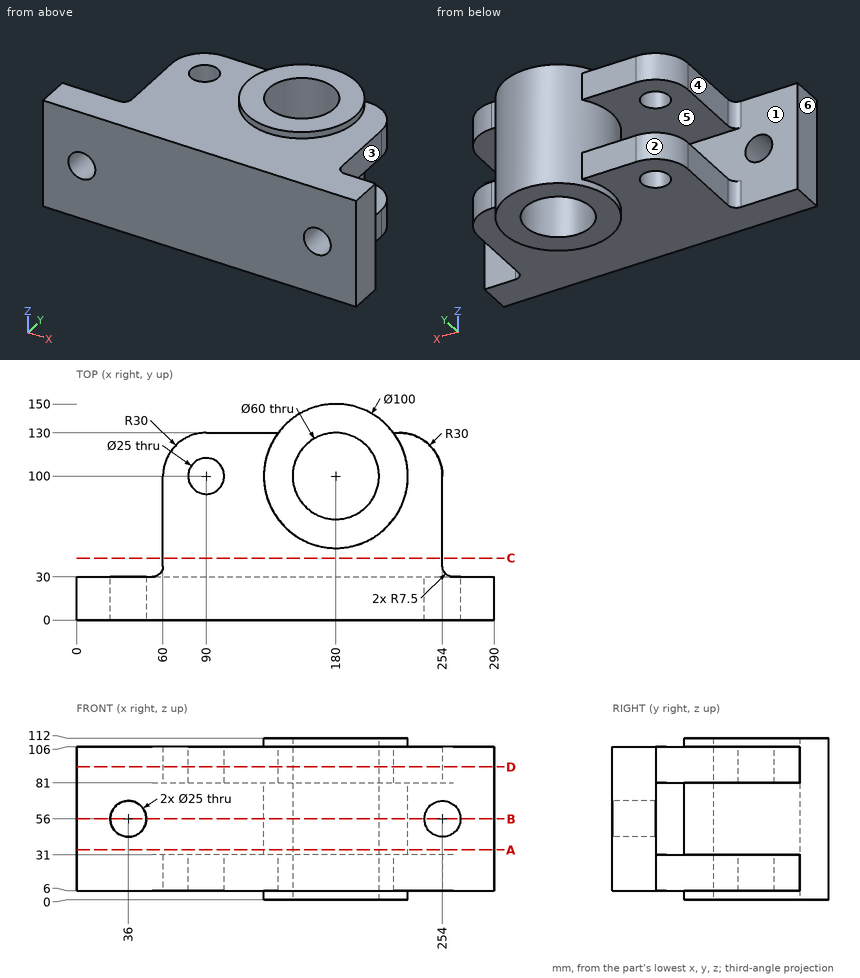
For this review, use the dimensioned drawing (mm, ordinates from the lowest corner) and the shaded views. A direction names the side the tool comes from. Give positions to 0.01 mm unless a question says otherwise; leave off trailing zeros. Order: outer loops, then holes, each group sorted by start corner. A loop starts at its lowest first (then second) coordinate and runs counter-clockwise, first axis right, second up.
1) Take a section at C-C (y = 43). Give the boundary of the cut face in (x, z), then the cut area to 3 significant figures.
2) Take a section at B-B (z = 56). Give the boundary of the cut face in (x, y), then the cut area to 3 significant figures.
3) Wall thickness on line 1 (Y direction, x = 180, z = 55); line 2 (Z direction, x = 113.5, y = 92.5); line 3 (Y direction, x = 90, z = 18): over which ranges is each line inside the solid? List them lowest first.
4) Take a section at A-A (z = 34.5). Give the boundary of the cut face in (x, y), then the cut area to 3 significant figures.
5) For the marked faces 4, 5 and 6, list the 3-axis set-ups (+Z, -Z, +X, -X, +Y, -Y) from which the entire face can be reached by the end or side of a thin tool; tool diameter is ignored.
6) Take a section at D-D (z = 92). Give the boundary of the cut face in (x, y), then the cut area to 3 significant figures.
7) Insertion check: pin 1 (4 mm diameter, centred on x = 79, z = 53, fed in from +Y); pin 2 (8 mm diameter, centred on x = 139.5, y = 23.5, fed in from -Z); pin 3 (20 mm diameter, centred on x = 117.5, z = 21.5, fed in from +Y). Each pin has a flat end and moves straight along its axis. Give the tip position at first contact, or say it passes through.
8) The part is to be moulded in two halves that separate along Y. For the marked faces 1, 2 and 3, say which applies: released by +Y, released by -Y, zero draft, split by the parting line, or undercut.
Derived:
1. outline: (60, 6) - (254, 6) - (254, 31) - (60, 31) - close; (60, 81) - (254, 81) - (254, 106) - (60, 106) - close
1. area: 9,700 mm2
2. outline: (0, 0) - (23.5, 0) - (23.5, 30) - (0, 30) - close; (48.5, 0) - (241.5, 0) - (241.5, 30) - (48.5, 30) - close; circle Ø100 at (180, 100); (266.5, 0) - (290, 0) - (290, 30) - (266.5, 30) - close; hole circle Ø60 at (180, 100)
2. area: 12,200 mm2
3. line 1: y = 0 to 30, 50 to 70, 130 to 150
3. line 2: z = 6 to 31, 81 to 106
3. line 3: y = 0 to 87.5, 112.5 to 130
4. outline: (0, 0) - (290, 0) - (290, 30) - (0, 30) - close; circle Ø100 at (180, 100); hole circle Ø60 at (180, 100)
4. area: 13,700 mm2
5. face 4: +Z, -Z, -X, +Y
5. face 5: none
5. face 6: +Z, -Z, -X, +Y, -Y
6. outline: (0, 0) - (290, 0) - (290, 30) - (261.5, 30) arc R7.5 cw to (254, 37.5) - (254, 100) arc R30 ccw to (224, 130) - (220, 130) arc R50 ccw to (140, 130) - (90, 130) arc R30 ccw to (60, 100) - (60, 37.5) arc R7.5 cw to (52.5, 30) - (0, 30) - close; hole circle Ø25 at (90, 100); hole circle Ø60 at (180, 100)
6. area: 25,500 mm2
7. pin 1: stops at y = 30
7. pin 2: stops at z = 6
7. pin 3: stops at y = 130
8. face 1: undercut
8. face 2: released by +Y
8. face 3: zero draft
